Part print with two shaded views. Sizes in mm from the minimum x, y, z corner. A direction names the side the tool comes from. Round coordinates to 2 decimals unless told otherwise and drop trailing zeros. Order: outer loops, then holes, each group sorted by start corner. A loop starts at its lowest first (then second) coordinate and runs counter-clockwise, first axis right, second up. Notation, with made-up numbers: (52, -17.75) - (76, -17.75) arc R28 ccw to (76, 19.25) - close; hole circle Ø1 at (60, 51). An arc over 180 degrees is marked (long way). Answer as CSV lines item,"result". Start each with the question number.
1. Band-saw the part on C-C on y = 4.5. List the corners of the cut face in (x, z), then the cut area to 3 significant figures.
2. 3-axis set-ups, long thin cutter, end or side, ignore diameter. For the marked faces 4, 5, 6 and 7: which of +Z, -Z, +X, -X, +Y, -Y reach the whole face in a straight line?
3. Band-saw the part on B-B on z = 26. List the corners of the cut face in (x, y), then the cut area to 3 significant figures.
4. Band-saw the part on D-D on y = 13.25. List the corners of the cut face in (x, z) (3 decimals), then the cut area to 3 significant figures.
5. Pull direction Z, two halves, no side cores. Call the marked faces 1, 2 and 3: released by +Z, released by -Z, zero draft, split by the parting line, or undercut.
6. Wall check: line 1 along Z through (x, y) = (26, 3); line 2 along Z through (x, y) = (26, 21); line 3 along Y through (x, z) = (48, 19). Give the ranges that are in metal, low to high. Write a range as [from, to].
7. Band-saw the part on A-A on x = 26. List the corners of the cut face in (y, z).
8. Pin check, flat tips, straight feed: pin 1 Ø5 at (x, y) = (22, 3.5) entering from -Z; pin 2 Ø1.5 at (y, z) = (9.5, 10) entering from +X; pin 3 Ø3 at (x, y) = (28, 19.5) entering from +Z. Stop position of each tip, or through.
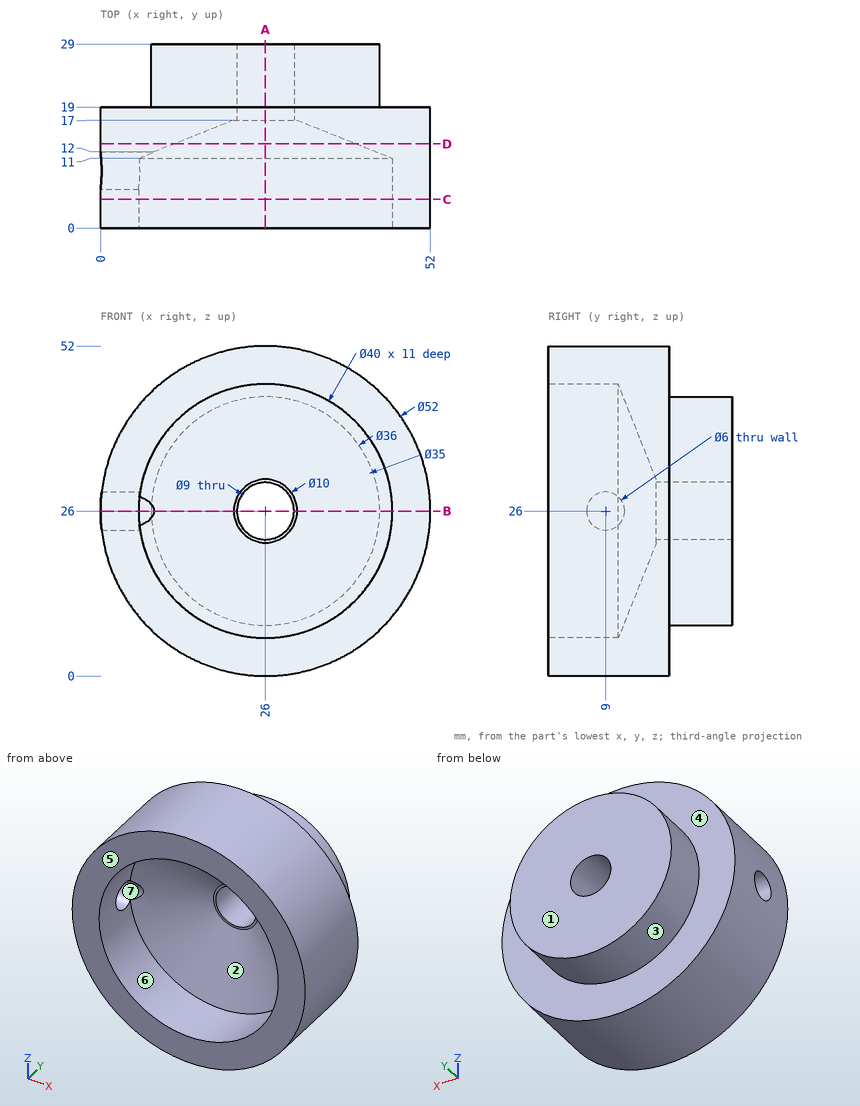
Reply:
1,outline,"circle Ø52 at (26, 26); hole circle Ø40 at (26, 26)"
1,area,"867 mm2"
2,face 4,"+Y"
2,face 5,"+Z, -Z, +X, -X, -Y"
2,face 6,"-Y"
2,face 7,"-X"
3,outline,"(0, 0) - (6, 0) - (6, 6) - (0, 6) - close; (0, 12) - (8.5, 12) - (21, 17) - (21.5, 17) - (21.5, 29) - (8, 29) - (8, 19) - (0, 19) - close; (30.5, 17) - (31, 17) - (46, 11) - (46, 0) - (52, 0) - (52, 19) - (44, 19) - (44, 29) - (30.5, 29) - close"
3,area,"613 mm2"
4,outline,"circle Ø52 at (26, 26); hole circle Ø28.75 at (26, 26)"
4,area,"1,470 mm2"
5,face 1,"zero draft"
5,face 2,"undercut"
5,face 3,"split by the parting line"
6,line 1,"z = [0, 6], [46, 52]"
6,line 2,"z = [8, 21.5], [30.5, 44]"
6,line 3,"y = [0, 19]"
7,outline,"(0, 0) - (19, 0) - (19, 8) - (29, 8) - (29, 21.5) - (17, 21.5) - (17, 21) - (11, 6) - (0, 6) - close; (0, 46) - (11, 46) - (17, 31) - (17, 30.5) - (29, 30.5) - (29, 44) - (19, 44) - (19, 52) - (0, 52) - close"
8,pin 1,"stops at z = 0.04"
8,pin 2,"stops at x = 47.06"
8,pin 3,"stops at z = 51.99"
